Source: three-view drawing plus pictorial views. Frame: mm from the lowest corner of the part. Coordinates: 2 decimals unless noted, no trailing zeros. Write each loop counter-clockwise with the first axis right and the second up, starting at its lowest first coordinate (ties: lowest second). Pieces come first, ordered by that corner, then holes. Notation, with made-up numbers: (-18.5, 1) -> (9.5, 1) arc R12 ccw to (9.5, 13) -> close; hole circle Ø5 at (15, -28). An arc over 180 degrees is marked (long way). One line per item, written item: value.
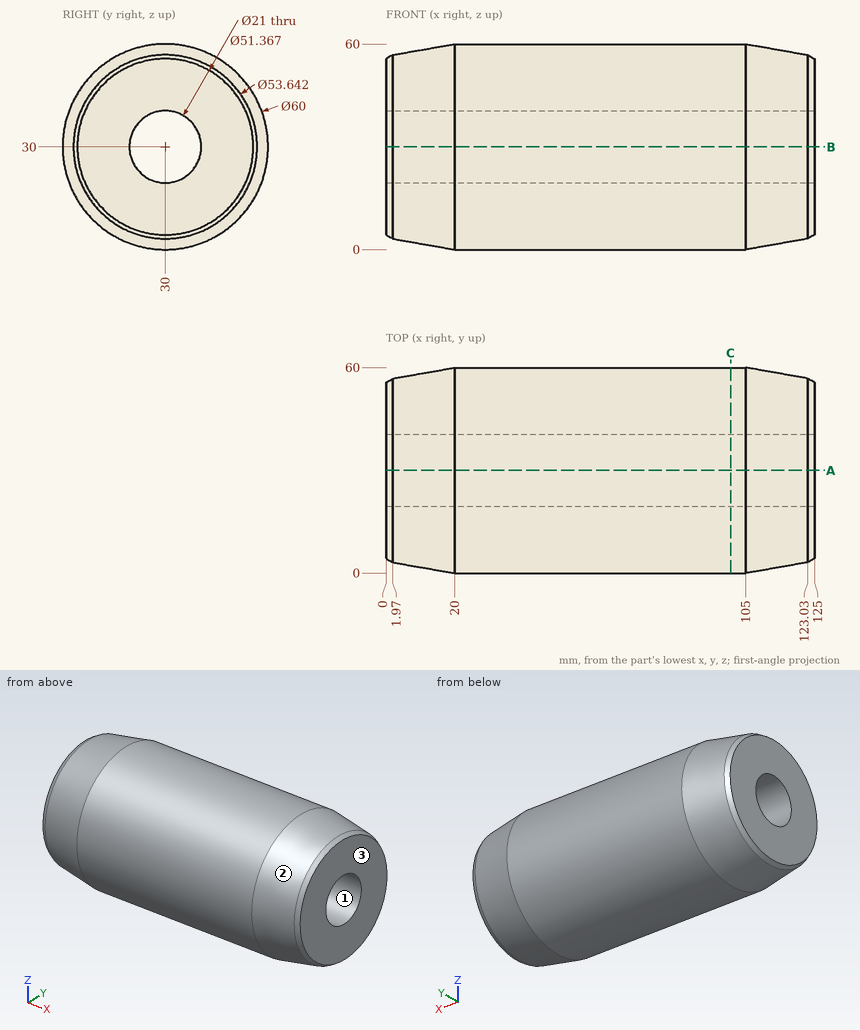
(1) First-contact query: pin 1 (1.5 mm diameter, centred on x = 74, z = 19.5, fed in from +Y); pin 2 (2 mm diameter, centred on x = 81.5, y = 41.5, fed in from +Z); pin 3 (2 mm diameter, centred on x = 71, z = 21.5, fed in from +Y). Flat tips, straight axial feed; report the tip coordinate or a pass-through.
Responses:
pin 1: stops at y = 58.37
pin 2: stops at z = 58.1
pin 3: stops at y = 59.05
(2) Section A-A (y = 30). Return the cut outline in (x, z), then the cut area to 3 significant figures.
Responses:
outline: (0, 4.32) -> (1.97, 3.18) -> (20, 0) -> (105, 0) -> (123.03, 3.18) -> (125, 4.32) -> (125, 19.5) -> (0, 19.5) -> close; (0, 40.5) -> (125, 40.5) -> (125, 55.68) -> (123.03, 56.82) -> (105, 60) -> (20, 60) -> (1.97, 56.82) -> (0, 55.68) -> close
area: 4,730 mm2
(3) Line query: line 1 (Y direction, x = 74, z = 30); line 2 (Z direction, x = 78.5, y = 38) (1 decimal); line 3 (Z direction, x = 103.5, y = 27). Output: solid intervals per line, ascending. Write a range as [from, to].
Responses:
line 1: y = [0, 19.5], [40.5, 60]
line 2: z = [1.1, 23.2], [36.8, 58.9]
line 3: z = [0.15, 19.94], [40.06, 59.85]
(4) Section C-C (x = 100.5). Return the cut outline in (y, z).
Responses:
outline: circle Ø60 at (30, 30); hole circle Ø21 at (30, 30)
(5) Pull-direction query (Z, two-part tool) for the marked faces 1, 2 and 3; classes: released by +Z, released by -Z, zero draft, split by the parting line, or undercut.
Responses:
face 1: undercut
face 2: split by the parting line
face 3: zero draft
